Answer from the drawing. Dimensions are ordinates in mm from the lowest x, y and z of the part. A direction names the side the tool comes from. Coordinates: 2 decimals unless noted, no trailing zeros. Write each loop counter-clockwise with the first axis right and the second up, starting at its lowest first coordinate (ties: lowest second). Pieces come first, ordered by that corner, then holes. Notation, with made-up numbers: (89, -1.5) - (128, -1.5) arc R20 cw to (128, 4.5) - close; hole circle Ø7 at (-3, -7). An arc over 180 degrees is marked (long way). Use one line per item in the form item = value. Start each with the question number.
Item 1: A cutting plane is placed at D-D (y = 54). Write down the section's boundary in (x, z).
Item 2: A cutting plane is placed at A-A (y = 544). Write down the section's boundary in (x, z), then the cut area to 3 significant figures.
Item 3: A cutting plane is placed at C-C (x = 180). Write down the section's boundary in (y, z).
Item 4: A cutting plane is placed at B-B (z = 140). Write down the section's boundary in (x, y), then the cut area to 3 significant figures.
Item 5: For the marked faces 1, 2 and 3, determine the directions among +Z, -Z, +X, -X, +Y, -Y from which every point of the face is accessible in a straight line to the end or side of a thin tool.
Item 6: Consider probe 1 along X at (y, z) = (693, 247); probe 2 along Z at (x, y) = (21, 705); probe 3 along X at (y, z) = (275, 142). Determine where each line is inside the solid, lowest interval first.
Item 7: Given pin 1 (5 mm diameter, centred on x = 97.5, z = 80, fed in from -Y); pin 2 (2 mm diameter, centred on x = 92.5, z = 150.5, fed in from +Y), each flat-ended and moving along its own axis, determine where each tip first touches the part or whether it passes through.
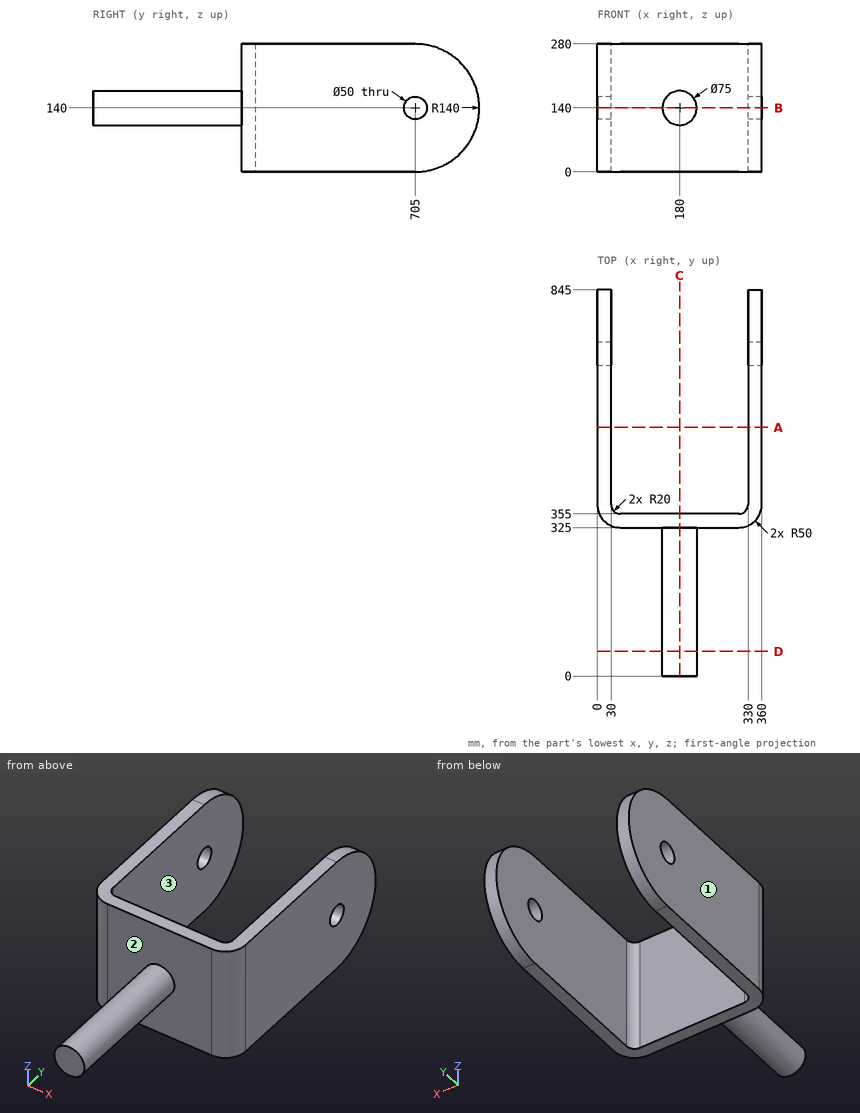
Answer:
q1.outline = circle Ø75 at (180, 140)
q2.outline = (0, 0) - (30, 0) - (30, 280) - (0, 280) - close; (330, 0) - (360, 0) - (360, 280) - (330, 280) - close
q2.area = 16,800 mm²
q3.outline = (0, 102.5) - (325, 102.5) - (325, 0) - (355, 0) - (355, 280) - (325, 280) - (325, 177.5) - (0, 177.5) - close
q4.outline = (0, 375) arc R50 ccw to (50, 325) - (142.5, 325) - (142.5, 0) - (217.5, 0) - (217.5, 325) - (310, 325) arc R50 ccw to (360, 375) - (360, 680) - (330, 680) - (330, 375) arc R20 cw to (310, 355) - (50, 355) arc R20 cw to (30, 375) - (30, 680) - (0, 680) - close; (0, 730) - (30, 730) - (30, 845) - (0, 845) - close; (330, 730) - (360, 730) - (360, 845) - (330, 845) - close
q4.area = 60,700 mm²
q5.face_1 = +Z, -Z, -X, +Y, -Y
q5.face_2 = -Y
q5.face_3 = +Z, -Z, +Y
q6.probe_1 = 0 to 30, 330 to 360
q6.probe_2 = 0 to 115, 165 to 280
q6.probe_3 = 142.55 to 217.45
q7.pin_1 = 325
q7.pin_2 = 355
